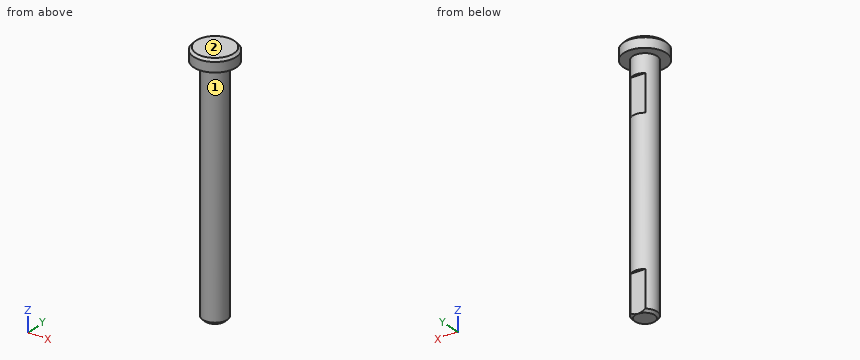
from build123d import *

# Parameters (mm, degrees)
SKETCH1_R           = 1
BOSS_EXTRUDE1_DEPTH = 9.75
SKETCH2_R           = 1.75
BOSS_EXTRUDE2_DEPTH = 1
CHAMFER1_SIZE       = 0.2
CUT_EXTRUDE1_START  = -3.2
CUT_EXTRUDE1_DEPTH  = 3.2
CUT_EXTRUDE2_DEPTH  = 1.5


with BuildPart() as part:
    # Sketch1 → Boss-Extrude1 (new, symmetric)
    with BuildSketch(Plane.XY):
        Circle(SKETCH1_R)
    extrude(amount=BOSS_EXTRUDE1_DEPTH, both=True)

    # Sketch2 → Boss-Extrude2 (add)
    with BuildSketch(Plane.XY.offset(9.75)):
        Circle(SKETCH2_R)
    extrude(amount=BOSS_EXTRUDE2_DEPTH)

    # Chamfer1
    chamfer1_edges = [part.edges().sort_by_distance(p)[0] for p in [
        (-1, 0, -9.75),
        (-1.75, 0, 10.75),
    ]]
    chamfer(chamfer1_edges, length=CHAMFER1_SIZE)

    # Sketch3 → Cut-Extrude1 (cut)
    with BuildSketch(Plane(origin=(0, 0, -9.75), x_dir=(-1, 0, 0), z_dir=(0, 0, -1)).offset(CUT_EXTRUDE1_START)):
        with BuildLine():
            Line((-0.6, 0.8), (0.6, 0.8))
            ThreePointArc((0.6, 0.8), (0, 1), (-0.6, 0.8))
        make_face()
    extrude(amount=CUT_EXTRUDE1_DEPTH, mode=Mode.SUBTRACT)

    # Sketch4 → Cut-Extrude2 (cut, symmetric)
    with BuildSketch(Plane(origin=(0, 0, 6.75), x_dir=(-1, 0, 0), z_dir=(0, 0, -1))):
        with BuildLine():
            Line((-0.6, 0.8), (0.6, 0.8))
            ThreePointArc((0.6, 0.8), (0, 1), (-0.6, 0.8))
        make_face()
    extrude(amount=CUT_EXTRUDE2_DEPTH, both=True, mode=Mode.SUBTRACT)


solid = part.part
Input: part model. Units: mm. Frame: model coordinates. Face numbers are marked on the shaded views. A direction names the side the tool comes from. Coordinates: 2 decimals unless noted, no trailing zeros. Order: outer loops, then holes, each group sorted by start corner. A loop starts at its lowest first (then second) coordinate and runs counter-clockwise, first axis right, second up. Notation, with made-up numbers: M -30,88 L 28,88 A25 cw 28,107 Z; hole C -32,81.25 d11. An arc over 180 degrees is marked long. Write item = value, one per line. Start each with the question number.
(1) Reachability of the marked faces 1 and 2 from +Z, -Z, +X, -X, +Y, -Y: full face, straight path, thin tool, end or side. Return the list, or none.
(2) Line query: line 1 along Z through (x, y) = (-1.2, 0.7); line 2 along X through (y, z) = (-0.8, -0.5); line 3 along Y through (x, z) = (0.1, -4.25). Output: solid intervals per line, ascending. Write a range as [from, to].
(3) First-contact query: P1, Ø1, axis at y = 1, z = -0.5, coming from the -X side; P2, Ø1, axis at x = 0, z = -8, coming from the +Y side. Flat tips, straight axial feed; report the tip coordinate or a pass-through.
(4) Section B-B on z = -6. Output: boundary loops of the cut face in (x, y).
(5) Section A-A on z = -8.25. Output: boundary loops of the cut face in (x, y), and give its area (3 significant figures).
Result set:
q1.face_1 = -Z
q1.face_2 = +Z, +X, -X, +Y, -Y
q2.line_1 = [9.75, 10.75]
q2.line_2 = [-0.6, 0.6]
q2.line_3 = [-0.99, 0.99]
q3.P1 = -0.87
q3.P2 = 0.8
q4.outline = C 0,0 d2
q5.outline = M -0.6,0.8 A1 ccw long 0.6,0.8 Z
q5.area = 2.98 mm²
